```python
from build123d import *

# Parameters (mm, degrees)
HEX_HEAD_DEPTH     = 20
SHANK_PROFILE_26_R = 13
SHANK_26X300_DEPTH = 300


with BuildPart() as part:
    # Hex Head Profile 35AF → Hex Head (new body)
    with BuildSketch(Plane(origin=(0, 0, 0), x_dir=(1, 0, 0), z_dir=(0, 1, 0))):
        Polygon((20.207259422, 0), (10.103629711, 17.5), (-10.103629711, 17.5), (-20.207259422, 0), (-10.103629711, -17.5), (10.103629711, -17.5), align=None)
    extrude(amount=HEX_HEAD_DEPTH)

    # Shank Profile Ø26 → Shank Ø26x300 (add)
    with BuildSketch(Plane.XZ):
        with Locations(Location((0, 0, 0), (0, 0, 270))):
            Circle(SHANK_PROFILE_26_R)
    extrude(amount=SHANK_26X300_DEPTH)

    # Head Chamfer Profile → Head Chamfer (revolve, cut)
    with BuildSketch(Plane.XY):
        with BuildLine():
            Line((18.207259422, 20), (20.207259422, 20))
            Line((20.207259422, 20), (20.207259422, 18))
            ThreePointArc((20.207259422, 18), (19.457751072, 19.25049165), (18.207259422, 20))
        make_face()
    revolve(axis=Axis((0, 0, 0), (0, 1, 0)), mode=Mode.SUBTRACT)


solid = part.part
```
Could you check a few things on this model? Use its own coordinates, in mm. A direction names the side the tool comes from. Round coordinates to 2 decimals unless told otherwise and drop trailing zeros. Loops run counter-clockwise (first coordinate to the right, second up) from the corner with the lowest first, then second, coordinate; pieces in that order, holes last. Notation, with made-up numbers: (-31, 80.25) - (22, 80.25) arc R16 ccw to (22, 101.25) - close; hole circle Ø2 at (29.25, -35). An arc over 180 degrees is marked (long way). Answer in a Markdown table with one row per item. Add a question column.
(1) If we section it at C-C (y = -174.5): Please give me the cut outline in (x, z).
(2) I need wall thicknesses on line 1 along Y through (x, z) = (-18, -0.5); line 2 along X through (y, z) = (7.5, 4.5); line 3 along Z through (x, y) = (-3, -33). Which ranges of each line are inside material? Lowest first, please.
(3) For faces 1 (the face through (-7.91, -147.9, 10.316)), 2 (the face through (0, 10, -17.5)), which set-ups out of +Z, -Z, +X, -X, +Y, -Y let a thin tool reach every point of the face, with its end or its side?
(4) If we section it at B-B (z = -7): Please give me the cut outline in (x, y).
(5) If we section it at A-A (x = 0): Please give me the cut outline in (y, z).
(6) I'm going to push flat-ended pins straight in: pin 1 (1 mm diameter, centred on y = -168, z = -0.5, fed in from -X); pin 2 (5 mm diameter, centred on x = -9, y = -145, fed in from +Z); pin 3 (4 mm diameter, centred on y = -203.5, z = -11, fed in from +X). Where does each tip first touch, or does it pass through?
Model answer:
| question | item | result |
|---|---|---|
| 1 | outline | circle Ø26 at (0, 0) |
| 2 | line 1 | y = 0 to 20 |
| 2 | line 2 | x = -17.61 to 17.61 |
| 2 | line 3 | z = -12.65 to 12.65 |
| 3 | face 1 | -Y |
| 3 | face 2 | -Z, +X, -X, +Y, -Y |
| 4 | outline | (-16.17, 0) - (-10.95, 0) - (-10.95, -300) - (10.95, -300) - (10.95, 0) - (16.17, 0) - (16.17, 20) - (-16.17, 20) - close |
| 5 | outline | (-300, -13) - (0, -13) - (0, -17.5) - (20, -17.5) - (20, 17.5) - (0, 17.5) - (0, 13) - (-300, 13) - close |
| 6 | pin 1 | stops at x = -13 |
| 6 | pin 2 | stops at z = 11.26 |
| 6 | pin 3 | stops at x = 9.38 |
